CAD build for the part. Positions are in the model's coordinates, mm. A direction names the side the tool comes from. Coordinates: 2 decimals unless noted, no trailing zeros. Order: outer loops, then holes, each group sorted by start corner. A loop starts at its lowest first (then second) coordinate and runs counter-clockwise, first axis right, second up. Notation, with made-up numbers: M -28.5,-36 L 15.5,-36 A26 cw 15.5,-9 Z; hole C 81,2 d8. An arc over 180 degrees is marked long. Write item = value, one per line. Start each with the question number.
```python
from build123d import *

# Parameters (mm, degrees)
C_FRAME_BODY_DEPTH        = 80
FRONT_BOSS_SKETCH_R       = 25
FRONT_BOSS_50_DEPTH       = 10
TOP_LUG_GUSSET_DEPTH      = 10
SKETCH3_3_R               = 20
TOP_LUG_RING_DEPTH        = 25
LOWER_RIB_REACH           = 169.929
LOWER_RIB_SKETCH_W        = 10
LOWER_RIB_SKETCH_H        = 9.5
RIB_EXTENSION_REACH       = 135.041
RIB_EXTENSION_SKETCH_W    = 10
RIB_EXTENSION_SKETCH_H    = 10
RIB_FILLET_R10_R          = 10
CONNECTING_STRAP_REACH    = 169.929
CONNECTING_STRAP_SKETCH_W = 15.505102572
CONNECTING_STRAP_SKETCH_H = 10
STRAP_RELIEF_CUT_DEPTH    = 25
FRONT_BORE_SKETCH_R       = 15
FRONT_BORE_30_DEPTH       = 25
TOP_HOLES_SKETCH_R        = 10
TOP_FACE_HOLES_DEPTH      = 25
LUG_BORE_DEPTH            = 157.604597634
LUG_CLAMP_SLOT_DEPTH      = 10
BASE_RELIEF_SKETCH_R      = 20
BASE_RELIEF_CUT_40_DEPTH  = 10


with BuildPart() as part:
    # C-Frame Profile Sketch → C-Frame Body (new body)
    with BuildSketch(Plane(origin=(0, 0, 0), x_dir=(0, 0, -1), z_dir=(1, 0, 0))):
        Polygon((0, 0), (-60, 0), (-60, 80), (-10, 80), (-10, 70), (-50, 70), (-50, 10), (0, 10), align=None)
    extrude(amount=-C_FRAME_BODY_DEPTH)

    # Front Boss Sketch → Front Boss _50 (add)
    with BuildSketch(Plane.XY.offset(60)):
        with Locations((-40, 40)):
            Circle(FRONT_BOSS_SKETCH_R)
    extrude(amount=FRONT_BOSS_50_DEPTH)

    # Top Lug Sketch → Top Lug Gusset (add)
    with BuildSketch(Plane(origin=(0, 0, 10), x_dir=(-1, 0, 0), z_dir=(0, 0, -1))):
        with BuildLine():
            ThreePointArc((60, 110), (34.899197777, 90.661390518), (22.601818332, 119.864242224))
            Line((22.601818332, 119.864242224), (0, 80))
            Line((0, 80), (80, 80))
            Line((80, 80), (57.398181668, 119.864242224))
            ThreePointArc((57.398181668, 119.864242224), (59.338609482, 115.100802223), (60, 110))
        make_face()
    extrude(amount=-TOP_LUG_GUSSET_DEPTH)

    # Sketch3_3 → Top Lug Ring (add)
    with BuildSketch(Plane(origin=(0, 0, 10), x_dir=(-1, 0, 0), z_dir=(0, 0, -1))):
        with Locations((40, 110)):
            Circle(SKETCH3_3_R)
    extrude(amount=-TOP_LUG_RING_DEPTH)

    # Lower Rib Sketch → Lower Rib (add, up to next)
    with BuildSketch(Plane.XY.offset(70), mode=Mode.PRIVATE) as lower_rib_sk1:
        with Locations((-40, 84.75)):
            Rectangle(LOWER_RIB_SKETCH_W, LOWER_RIB_SKETCH_H)
    lower_rib_tool1 = extrude(lower_rib_sk1.sketch, amount=-LOWER_RIB_REACH, mode=Mode.PRIVATE) - part.part
    add(lower_rib_tool1.solids().sort_by_distance((-40, 84.75, 70))[0])

    # Rib Extension Sketch → Rib Extension (add, up to next)
    with BuildSketch(Plane.XZ.offset(-80), mode=Mode.PRIVATE) as rib_extension_sk1:
        with Locations((-40, 65)):
            Rectangle(RIB_EXTENSION_SKETCH_W, RIB_EXTENSION_SKETCH_H)
    rib_extension_tool1 = extrude(rib_extension_sk1.sketch, amount=RIB_EXTENSION_REACH, mode=Mode.PRIVATE) - part.part
    add(rib_extension_tool1.solids().sort_by_distance((-40, 80, 65))[0])

    # Rib Fillet R10
    rib_fillet_r10_edges = [part.edges().sort_by_distance(p)[0] for p in [
        (-40, 89.5, 70),
    ]]
    fillet(rib_fillet_r10_edges, radius=RIB_FILLET_R10_R)

    # Connecting Strap Sketch → Connecting Strap (add, up to next)
    with BuildSketch(Plane.XY.offset(70), mode=Mode.PRIVATE) as connecting_strap_sk1:
        with Locations((-7.752551286, 40)):
            Rectangle(CONNECTING_STRAP_SKETCH_W, CONNECTING_STRAP_SKETCH_H)
    connecting_strap_tool1 = extrude(connecting_strap_sk1.sketch, amount=-CONNECTING_STRAP_REACH, mode=Mode.PRIVATE) - part.part
    # Connecting Strap Sketch → Connecting Strap (add, up to next)
    with BuildSketch(Plane.XY.offset(70), mode=Mode.PRIVATE) as connecting_strap_sk2:
        with Locations((-72.247448714, 40)):
            Rectangle(CONNECTING_STRAP_SKETCH_W, CONNECTING_STRAP_SKETCH_H)
    connecting_strap_tool2 = extrude(connecting_strap_sk2.sketch, amount=-CONNECTING_STRAP_REACH, mode=Mode.PRIVATE) - part.part
    add(connecting_strap_tool1.solids().sort_by_distance((-7.752551, 40, 70))[0])
    add(connecting_strap_tool2.solids().sort_by_distance((-72.247449, 40, 70))[0])

    # Strap Relief Sketch → Strap Relief Cut (cut)
    with BuildSketch(Plane(origin=(0, 45, 0), x_dir=(1, 0, 0), z_dir=(0, 1, 0))):
        Polygon((-15.505102572, -70), (0, -60), (0, -70), align=None)
        Polygon((-80, -60), (-64.494897428, -70), (-80, -70), align=None)
    extrude(amount=-STRAP_RELIEF_CUT_DEPTH, mode=Mode.SUBTRACT)

    # Front Bore Sketch → Front Bore _30 (cut)
    with BuildSketch(Plane.XY.offset(70)):
        with Locations((-40, 40)):
            Circle(FRONT_BORE_SKETCH_R)
    extrude(amount=-FRONT_BORE_30_DEPTH, mode=Mode.SUBTRACT)

    # Top Holes Sketch → Top Face Holes (cut)
    with BuildSketch(Plane(origin=(0, 80, 0), x_dir=(1, 0, 0), z_dir=(0, 1, 0))):
        with Locations(Location((-20, -35, 0), (0, 0, 270))):
            Circle(TOP_HOLES_SKETCH_R)
        with Locations(Location((-60, -35, 0), (0, 0, 270))):
            Circle(TOP_HOLES_SKETCH_R)
    extrude(amount=-TOP_FACE_HOLES_DEPTH, mode=Mode.SUBTRACT)

    # Lug Bore and Slot Sketch → Lug Bore (cut, through all)
    with BuildSketch(Plane.XY.offset(35)):
        with BuildLine():
            ThreePointArc((-37.5, 119.682458366), (-40, 120), (-42.5, 119.682458366))
            Line((-42.5, 119.682458366), (-37.5, 119.682458366))
        make_face()
        with BuildLine():
            Line((-37.5, 119.682458366), (-42.5, 119.682458366))
            ThreePointArc((-42.5, 119.682458366), (-46.123724357, 102.09430585), (-30, 110))
            ThreePointArc((-30, 110), (-32.09430585, 116.123724357), (-37.5, 119.682458366))
        make_face()
        with BuildLine():
            ThreePointArc((-37.5, 119.682458366), (-40, 120), (-42.5, 119.682458366))
            Line((-42.5, 119.682458366), (-37.5, 119.682458366))
        make_face()
        with BuildLine():
            Line((-37.5, 119.682458366), (-42.5, 119.682458366))
            ThreePointArc((-42.5, 119.682458366), (-46.123724357, 102.09430585), (-30, 110))
            ThreePointArc((-30, 110), (-32.09430585, 116.123724357), (-37.5, 119.682458366))
        make_face()
    extrude(amount=-LUG_BORE_DEPTH, mode=Mode.SUBTRACT)

    # Sketch14_3 → Lug Clamp Slot (cut)
    with BuildSketch(Plane.XY.offset(35)):
        with BuildLine():
            Line((-42.5, 129.843134833), (-42.5, 119.682458366))
            ThreePointArc((-42.5, 119.682458366), (-40, 120), (-37.5, 119.682458366))
            Line((-37.5, 119.682458366), (-37.5, 129.843134833))
            ThreePointArc((-37.5, 129.843134833), (-40, 130), (-42.5, 129.843134833))
        make_face()
    extrude(amount=-LUG_CLAMP_SLOT_DEPTH, mode=Mode.SUBTRACT)

    # Base Relief Sketch → Base Relief Cut _40 (cut)
    with BuildSketch(Plane(origin=(0, 10, 0), x_dir=(1, 0, 0), z_dir=(0, 1, 0))):
        with Locations((-40, 0)):
            Circle(BASE_RELIEF_SKETCH_R)
    extrude(amount=-BASE_RELIEF_CUT_40_DEPTH, mode=Mode.SUBTRACT)


solid = part.part
```
1. Slice it at D-D (x = -13.5). Write the cut outline in (y, z).
2. 3-axis set-ups, long thin cutter, end or side, ignore diameter. For faces 1 (the flat face through (-11, 45, 63)), 2 (the flat face through (-39, 94, 10)), 3 (the flat face through (-31, 115, 35)), 4 (the flat face through (-40, 89.5, 40)), 5 (the flat face through (-39, 10, 31)): which of +Z, -Z, +X, -X, +Y, -Y reach the whole face in a straight line?
3. Flat gauge pins, fed straight in: pin 1 (8 mm diameter, centred on x = -9.5, z = 62.5, fed in from +Y); pin 2 (11 mm diameter, centred on y = 124, z = 31, fed in from +X); pin 3 (12 mm diameter, centred on x = -40, y = 110, fed in from -Z); pin 4 (4 mm diameter, centred on x = -56.5, y = 80.5, fed in from -Z). Where does each tip first touch, or does it go through?
4. Probe L1, parallel to X at y = 77, z = 35; L2, parallel to Y at x = -40, z = 20.5; L3, parallel to X at y = 110, z = 29.25. List the from-to ranges inside material, lowest first.
5. Mould opens along Y. For faces 6 (the flat face through (-45, 83, 50)), 7 (the cylindrical face through (-40, 15, 65)), 8 (the flat face through (-68.86, 99.65, 14.93)) say: released by +Y, released by -Y, zero draft, split by the parting line, or undercut.
6. Slice it at B-B (y = 112). Write the cut outline in (x, z).
7. Slice it at A-A (x = -40). Write the cut outline in (y, z), plus the area to 3 significant figures.
8. Slice it at C-C (z = 26.5). Write the cut outline in (x, y).
Calculated:
q1.outline = M 0,0 L 10,0 L 10,50 L 70,50 L 70,42.6 L 80,42.6 L 80,60 L 45,60 L 45,68.71 L 35,68.71 L 35,60 L 0,60 Z; M 70,10 L 103.81,10 L 103.81,20 L 80,20 L 80,27.4 L 70,27.4 Z
q2.face_1 = +Z, +X, +Y
q2.face_2 = -Z, +X, -X, +Y
q2.face_3 = +Z, +X, -X, +Y
q2.face_4 = +Z, +X, -X
q2.face_5 = -Z, +X, -X
q3.pin_1 = 80
q3.pin_2 = -21.9
q3.pin_3 = through
q3.pin_4 = 10
q4.L1 = -80 to -70, -50 to -30, -10 to 0
q4.L2 = 0 to 10, 70 to 89.5, 90 to 100, 120 to 130
q4.L3 = -60 to -50, -30 to -20
q5.face_6 = undercut
q5.face_7 = released by -Y
q5.face_8 = released by +Y
q6.outline = M -61.86,10 L -49.8,10 L -49.8,35 L -59.9,35 L -59.9,20 L -61.86,20 Z; M -30.2,10 L -18.14,10 L -18.14,20 L -20.1,20 L -20.1,35 L -30.2,35 Z
q7.outline = M 0,20 L 10,20 L 10,50 L 25,50 L 25,70 L 15,70 L 15,60 L 0,60 Z; M 55,50 L 70,50 L 70,10 L 100,10 L 100,35 L 90,35 L 90,20 L 89.5,20 L 89.5,60 A10 ccw 79.5,70 L 55,70 Z; M 120,10 L 130,10 L 130,25 L 120,25 Z
q7.area = 2,500 mm²
q8.outline = M -80,0 L 0,0 L 0,10 L -80,10 Z; M -80,70 L -65.27,70 L -65.27,80 L -80,80 Z; M -54.73,70 L -25.27,70 L -25.27,80 L -35,80 L -35,89.5 L -45,89.5 L -45,80 L -54.73,80 Z; M -42.5,119.68 L -42.5,129.84 A20 ccw long -37.5,129.84 L -37.5,119.68 A10 cw long Z; M -14.73,70 L 0,70 L 0,80 L -14.73,80 Z
